Could you check a few things on this model? Use its own coordinates, in mm. A direction names the side the tool comes from. Give positions to 0.01 mm unless a question says otherwise; leave off trailing zeros. Loops run counter-clockwise (first coordinate to the right, second up) from the corner with the lowest first, then second, coordinate; pieces in that order, holes last. Notation, with made-up numbers: M 60,24.25 L 88,24.25 A21 cw 88,32.25 Z; hole C 45.25,-6.5 d5. An arc over 180 degrees is marked long. Return JSON: item names as keys, results as strings. Group by question number.
1. If we mould it in two halves opening along Y, with no side actions, what happens to faces 5 (the flat face through (-25, 33, 17)), 6 (the flat face through (-47, 35, 19)), 7 (the cylindrical face through (15.242, 13.998, 10.488)), 8 (the flat face through (-1, 17, 25))? For each: +Y half, -Y half, draft (parallel to the pull), parting line (faces both ways), or undercut.
2. For faces 1 (the flat face through (40, 32, 16)), 2 (the cylindrical face through (-15.386, 26.128, 14.465)), 3 (the flat face through (30, 24, -5)), 4 (the flat face through (2.63, 5.59, 5.91)), which set-ups out of +Z, -Z, +X, -X, +Y, -Y let a thin tool reach every point of the face, with its end or its side?
3. Please list where these lines run through material, in increasing order: line 1 (Y direction, x = -20, z = 18.5); line 2 (Y direction, x = -20, z = 16.5); line 3 (Z direction, x = 36, y = 47.5).
4. If we section it at A-A (z = 21.5): Write out the boundary of the cut face in (x, y).
5. If we section it at D-D (x = -2): Write out the boundary of the cut face in (y, z).
6. If we section it at B-B (x = -20): Write out the boundary of the cut face in (y, z), plus the area to 3 significant figures.
7. If we section it at C-C (y = 53.5): Write out the boundary of the cut face in (x, z), plus the area to 3 significant figures.
8. For pin 1 (3 mm diameter, centred on x = 15, y = 32.5, fed in from -Z); pin 2 (2.5 mm diameter, centred on y = 43.5, z = 19, fed in from +X); pin 3 (1.5 mm diameter, centred on x = -48.5, z = 18, fed in from -Y); pin 4 (6 mm diameter, centred on y = 23.5, z = -16.5, fed in from +X), each with a flat end and sliding along its axis, tell me the tip position at first contact or that it passes through.
```python
from build123d import *

# Parameters (mm, degrees)
BASE_BLOCK_DEPTH         = 63
CORNER_NOTCH_DEPTH       = 63
SIDE_POCKET_SKETCH_W     = 20
SIDE_POCKET_SKETCH_H     = 3.232862168
SIDE_POCKET_DEPTH        = 9
POCKET_SLOT_SKETCH_W     = 40
POCKET_SLOT_SKETCH_H     = 50
POCKET_SLOT_DEPTH        = 15
CIRCULAR_RECESS_SKETCH_R = 25
CIRCULAR_RECESS_DEPTH    = 13
PIN_BASE_20_SKETCH_R     = 10
PIN_BASE_20_DEPTH        = 5
PIN_10_SKETCH_R          = 5
PIN_10_DEPTH             = 8
RECESS_OPENING_DEPTH     = 13
THROUGH_SLOT_SKETCH_W    = 10
THROUGH_SLOT_SKETCH_H    = 12
THROUGH_SLOT_DEPTH       = 117
PROFILE_CUT_DEPTH        = 117
THROUGH_HOLE_10_SKETCH_R = 5
THROUGH_HOLE_10_DEPTH    = 117
CORNER_V_NOTCH_DEPTH     = 117


with BuildPart() as part:
    # Base Block Sketch → Base Block (new body)
    with BuildSketch(Plane(origin=(0, 0, 0), x_dir=(1, 0, 0), z_dir=(0, 1, 0))):
        Polygon((50, 0), (50, 25), (-50, 25), (-50, -25), (50, -25), align=None)
    extrude(amount=BASE_BLOCK_DEPTH)

    # Corner Notch Sketch → Corner Notch (cut)
    with BuildSketch(Plane.XY.offset(25)):
        with BuildLine():
            Line((35, 0), (22.104816934, 11.471476847))
            ThreePointArc((22.104816934, 11.471476847), (15.135621173, 13.994794618), (8.343659927, 11.027289849))
            Line((8.343659927, 11.027289849), (-3.246679913, 0))
            Line((-3.246679913, 0), (35, 0))
        make_face()
    extrude(amount=-CORNER_NOTCH_DEPTH, mode=Mode.SUBTRACT)

    # Side Pocket Sketch → Side Pocket (cut)
    with BuildSketch(Plane.XY.offset(25)):
        with BuildLine():
            ThreePointArc((30, 35), (35.857864376, 20.857864376), (50, 15))
            Line((50, 15), (50, 35))
            Line((50, 35), (50, 63))
            Line((50, 63), (30, 63))
            Line((30, 63), (30, 48))
            Line((30, 48), (30, 35))
        make_face()
        with Locations((40, 64.616431084)):
            Rectangle(SIDE_POCKET_SKETCH_W, SIDE_POCKET_SKETCH_H)
    extrude(amount=-SIDE_POCKET_DEPTH, mode=Mode.SUBTRACT)

    # Pocket Slot Sketch → Pocket Slot (cut)
    with BuildSketch(Plane(origin=(0, 63, 0), x_dir=(1, 0, 0), z_dir=(0, 1, 0))):
        with Locations((30, 0)):
            Rectangle(POCKET_SLOT_SKETCH_W, POCKET_SLOT_SKETCH_H)
    extrude(amount=-POCKET_SLOT_DEPTH, mode=Mode.SUBTRACT)

    # Circular Recess Sketch → Circular Recess (cut)
    with BuildSketch(Plane.XY.offset(25)):
        with Locations((-20, 35)):
            Circle(CIRCULAR_RECESS_SKETCH_R)
    extrude(amount=-CIRCULAR_RECESS_DEPTH, mode=Mode.SUBTRACT)

    # Pin Base Ø20 Sketch → Pin Base Ø20 (add)
    with BuildSketch(Plane.XY.offset(12)):
        with Locations((-20, 35)):
            Circle(PIN_BASE_20_SKETCH_R)
    extrude(amount=PIN_BASE_20_DEPTH)

    # Pin Ø10 Sketch → Pin Ø10 (add)
    with BuildSketch(Plane.XY.offset(17)):
        with Locations((-20, 35)):
            Circle(PIN_10_SKETCH_R)
    extrude(amount=PIN_10_DEPTH)

    # Recess Opening Sketch → Recess Opening (cut)
    with BuildSketch(Plane.XY.offset(25)):
        with BuildLine():
            Line((-45, 35), (-50, 35))
            Line((-50, 35), (-50, 10))
            ThreePointArc((-50, 10), (-42.09430585, 11.282917549), (-35, 15))
            ThreePointArc((-35, 15), (-42.360679775, 23.819660113), (-45, 35))
        make_face()
    extrude(amount=-RECESS_OPENING_DEPTH, mode=Mode.SUBTRACT)

    # Through Slot Sketch → Through Slot (cut)
    with BuildSketch(Plane(origin=(0, 63, 0), x_dir=(1, 0, 0), z_dir=(0, 1, 0))):
        with Locations((5, 19)):
            Rectangle(THROUGH_SLOT_SKETCH_W, THROUGH_SLOT_SKETCH_H)
    extrude(amount=-THROUGH_SLOT_DEPTH, mode=Mode.SUBTRACT)

    # Profile Cut Sketch → Profile Cut (cut)
    with BuildSketch(Plane(origin=(0, 48, 0), x_dir=(1, 0, 0), z_dir=(0, 1, 0))):
        Polygon((20, 5), (50, 5), (50, 25), (10, 25), (10, 5), align=None)
    extrude(amount=-PROFILE_CUT_DEPTH, mode=Mode.SUBTRACT)

    # Through Hole Ø10 Sketch → Through Hole Ø10 (cut)
    with BuildSketch(Plane(origin=(0, 63, 0), x_dir=(1, 0, 0), z_dir=(0, 1, 0))):
        with Locations(Location((-11, 5, 0), (0, 0, 270))):
            Circle(THROUGH_HOLE_10_SKETCH_R)
    extrude(amount=-THROUGH_HOLE_10_DEPTH, mode=Mode.SUBTRACT)

    # Corner V-Notch Sketch → Corner V-Notch (cut)
    with BuildSketch(Plane.ZY.offset(50)):
        Polygon((-25, 63), (-25, 45), (-18.448535783, 63), align=None)
    extrude(amount=-CORNER_V_NOTCH_DEPTH, mode=Mode.SUBTRACT)


solid = part.part
```
Answer:
{
 "1": {"face 5": "undercut", "face 6": "undercut", "face 7": "-Y half", "face 8": "draft"},
 "2": {"face 1": "+Z, +X, +Y", "face 2": "+Z", "face 3": "-Z, +X, +Y, -Y", "face 4": "+Z, -Z, -Y"},
 "3": {"line 1": "y = 0 to 10, 30 to 40, 60 to 63", "line 2": "y = 0 to 10, 25 to 45, 60 to 63", "line 3": "z = -5 to 16"},
 "4": {"outline": "M -50,0 L -3.25,0 L 8.34,11.03 A10 cw 22.1,11.47 L 35,0 L 50,0 L 50,15 A20 cw 30,35 L 30,48 L 10,48 L 10,63 L -50,63 L -50,35 L -45,35 A25 cw long -35,15 A25 cw -50,10 Z; C -20,35 d10"},
 "5": {"outline": "M 1.19,-25 L 45,-25 L 63,-18.45 L 63,25 L 52.35,25 L 52.35,12 L 17.65,12 L 17.65,25 L 1.19,25 Z"},
 "6": {"outline": "M 0,-25 L 45,-25 L 63,-18.45 L 63,25 L 60,25 L 60,12 L 45,12 L 45,17 L 40,17 L 40,25 L 30,25 L 30,17 L 25,17 L 25,12 L 10,12 L 10,25 L 0,25 Z", "area": "2,620 mm²"},
 "7": {"outline": "M -50,-21.91 L 0,-21.91 L 0,-13 L 10,-13 L 10,25 L -3.18,25 L -3.18,12 L -36.82,12 L -36.82,25 L -50,25 Z; hole C -11,-5 d10", "area": "2,210 mm²"},
 "8": {"pin 1": "stops at z = -5", "pin 2": "stops at x = 30", "pin 3": "stops at y = 0", "pin 4": "stops at x = 0"}
}
